Could you check a few things on this model? Use its own coordinates, in mm. A direction names the side the tool comes from. Round coordinates to 2 decimals unless told otherwise and drop trailing zeros. Write each loop counter-clockwise with the first axis right and the second up, starting at its lowest first coordinate (ties: lowest second). Pieces come first, ordered by that corner, then holes. Notation, with made-up numbers: (50, -1) -> (93, -1) arc R19 cw to (93, 29) -> close; hole circle Ø11 at (15, 53). An arc over 180 degrees is marked (long way). Answer in a Markdown table with one row per item.
from build123d import *

# Parameters (mm, degrees)
BOSS_EXTRUDE1_DEPTH = 660.4


with BuildPart() as part:
    # Sketch1 → Boss-Extrude1 (new, symmetric)
    with BuildSketch(Plane.XY):
        with BuildLine():
            Line((0, 50), (0, 0))
            Line((0, 0), (50, 0))
            Line((50, 0), (50, 4))
            ThreePointArc((50, 4), (49.414213562, 5.414213562), (48, 6))
            Line((48, 6), (11.5, 6))
            ThreePointArc((11.5, 6), (7.610912703, 7.610912703), (6, 11.5))
            Line((6, 11.5), (6, 48))
            ThreePointArc((6, 48), (5.414213562, 49.414213562), (4, 50))
            Line((4, 50), (0, 50))
        make_face()
    extrude(amount=BOSS_EXTRUDE1_DEPTH, both=True)


solid = part.part
1) For pin 1 (12 mm diameter, centred on y = 28.5, z = -287.5, fed in from -X); pin 2 (18 mm diameter, centred on y = 33.5, z = 0.5, fed in from +X); pin 3 (18 mm diameter, centred on x = 29.5, z = 150, fed in from +Y), each with a flat end and sliding along its axis, tell me the tip position at first contact or that it passes through.
Findings:
| item | result |
|---|---|
| pin 1 | stops at x = 0 |
| pin 2 | stops at x = 6 |
| pin 3 | stops at y = 6 |
2) Imagine slicing it at B-B, the plane x = 24. Please give me the cut outline in (y, z).
Findings:
| item | result |
|---|---|
| outline | (0, -660.4) -> (6, -660.4) -> (6, 660.4) -> (0, 660.4) -> close |
3) For faces 1 (the face through (5, 16, 660.4)), 2 (the face through (6, 29, 9)), which set-ups out of +Z, -Z, +X, -X, +Y, -Y let a thin tool reach every point of the face, with its end or its side?
Findings:
| item | result |
|---|---|
| face 1 | +Z, +X, -X, +Y, -Y |
| face 2 | +Z, -Z, +X, +Y |
4) Please list where these lines run through material, in increasing order: line 1 (X direction, y = 23, z = 134); line 2 (X direction, y = 4.5, z = -586.5).
Findings:
| item | result |
|---|---|
| line 1 | x = 0 to 6 |
| line 2 | x = 0 to 49.94 |
5) Imagine slicing it at A-A, the plane z = 275. Please give me the cut outline in (x, y).
Findings:
| item | result |
|---|---|
| outline | (0, 0) -> (50, 0) -> (50, 4) arc R2 ccw to (48, 6) -> (11.5, 6) arc R5.5 cw to (6, 11.5) -> (6, 48) arc R2 ccw to (4, 50) -> (0, 50) -> close |
